Source: CAD feature listing. Evaluate the final solid. Frame: model axes, mm. A direction names the side the tool comes from. Coordinates: 2 decimals unless noted, no trailing zeros. Write each loop counter-clockwise with the first axis right and the second up, starting at its lowest first coordinate (ties: lowest second). Pieces come first, ordered by that corner, then holes. Notation, with made-up numbers: (2, 22) -> (14, 22) arc R30 ccw to (14, 55) -> close; hole circle Ø5 at (29.25, -3.75). An arc over 180 degrees is marked (long way). One line per item, written item: value. Start each with the question number.
1. Section query A-A, the plane y = 127.5. Output: boundary loops of the cut face in (x, z), and give its area (3 significant figures).
2. First-contact query: P1, Ø1.3, axis at y = -17.5, z = 23, coming from the -X side; P2, Ø2, axis at y = -14.5, z = 23.5, coming from the +X side; P3, Ø4.5, axis at x = 36.77, z = 36.77, coming from the -Y side. Flat tips, straight axial feed; report the tip coordinate or a pass-through.
3. Mould query, pull axis X, two halves, no side actions, for faces 1 (the flat face through (-1, 24, 45)), 2 (the conical face through (-36.75, 18.241, -37.203)), 3 (the cylindrical face through (-17.235, 104.695, 41.569)), 4 (the conical face through (-37.203, 18.241, 36.75)). Classes: released by +X, released by -X, zero draft, split by the parting line, or undercut.
4. Access query for faces 5 (the flat face through (-30, 163, 13)), 6 (the flat face through (0, -18, 22.5)), 7 (the flat face through (-34, 48, 34)), 8 (the flat face through (-34, 48, -34)). Directions: +Z, -Z, +X, -X, +Y, -Y. A direction counts if a zero-diameter tool reaches every point of the face in a straight line with its end or side. Return the directions, or none.
5. Line query: line 1 (Y direction, x = 25, z = 14); line 2 (Y direction, x = 29.5, z = -32); line 3 (X direction, y = 130, z = 0.5). Output: solid intervals per line, ascending.
from build123d import *

# Parameters (mm, degrees)
SKETCH_1_W               = 90
SKETCH_1_H               = 90
EXTRUDE_1_DEPTH          = 43
SKETCH_2_R               = 18
EXTRUDE_2_DEPTH          = 3
SKETCH_3_R               = 7.5
EXTRUDE_3_DEPTH          = 29
CUT_EXTRUDE_1_DEPTH      = 3
PATTERN_CIRCULAR_1_COUNT = 4
SKETCH_8_R               = 45
EXTRUDE_4_DEPTH          = 120
SKETCH_9_R               = 32.5
EXTRUDE_5_DEPTH          = 5
SKETCH_10_W              = 90
SKETCH_10_H              = 90
EXTRUDE_6_DEPTH          = 5
FILLET_1_R               = 5
FILLET_2_R               = 2


with BuildPart() as part:
    # 草图1 → 凸台-拉伸1 (new body)
    with BuildSketch(Plane(origin=(0, 0, 0), x_dir=(1, 0, 0), z_dir=(0, 1, 0))):
        Rectangle(SKETCH_1_W, SKETCH_1_H)
    extrude(amount=EXTRUDE_1_DEPTH)

    # 草图2 → 凸台-拉伸2 (add)
    with BuildSketch(Plane.XZ):
        with Locations(Location((0, 18, 0), (0, 0, 90))):
            Circle(SKETCH_2_R)
    extrude(amount=EXTRUDE_2_DEPTH)

    # 草图3 → 凸台-拉伸3 (add)
    with BuildSketch(Plane.XZ.offset(3)):
        with Locations(Location((0, 18, 0), (0, 0, 90))):
            Circle(SKETCH_3_R)
    extrude(amount=EXTRUDE_3_DEPTH)

    # 草图4 → 切除-拉伸1 (cut)
    with BuildSketch(Plane.XY.offset(25.5)):
        with BuildLine():
            Line((-2.5, -7), (-2.5, -32))
            Line((-2.5, -32), (2.5, -32))
            Line((2.5, -32), (2.5, -7))
            ThreePointArc((2.5, -7), (0, -4.5), (-2.5, -7))
        make_face()
    extrude(amount=-CUT_EXTRUDE_1_DEPTH, mode=Mode.SUBTRACT)

    # 草图6 → M6x1.0 螺纹孔1 (revolve, cut)
    with BuildSketch(Plane(origin=(36.769552622, 0, 36.769552622), x_dir=(0, 0, -1), z_dir=(1, 0, 0))):
        Polygon((0, 0), (0, 18.502151548), (2.5, 17), (2.5, 0), align=None)
    m6x1_0_1 = revolve(axis=Axis((36.769552622, -6.35, 36.769552622), (0, 1, 0)), mode=Mode.SUBTRACT)

    # 阵列(圆周)1: M6x1.0 螺纹孔1 ×4 about axis
    pattern_circular_1_axis = Axis((0, 0, 0), (0, 1, 0))
    for i in range(1, PATTERN_CIRCULAR_1_COUNT):
        add(m6x1_0_1.rotate(pattern_circular_1_axis, i * 360 / PATTERN_CIRCULAR_1_COUNT), mode=Mode.SUBTRACT)

    # 草图8 → 凸台-拉伸4 (add)
    with BuildSketch(Plane(origin=(0, 43, 0), x_dir=(1, 0, 0), z_dir=(0, 1, 0))):
        with Locations(Location((0, 0, 0), (0, 0, 270))):
            Circle(SKETCH_8_R)
    extrude(amount=EXTRUDE_4_DEPTH)

    # 草图9 → 凸台-拉伸5 (add)
    with BuildSketch(Plane(origin=(0, 163, 0), x_dir=(1, 0, 0), z_dir=(0, 1, 0))):
        with Locations(Location((0, 0, 0), (0, 0, 270))):
            Circle(SKETCH_9_R)
    extrude(amount=EXTRUDE_5_DEPTH)

    # 草图10 → 凸台-拉伸6 (add)
    with BuildSketch(Plane(origin=(0, 43, 0), x_dir=(1, 0, 0), z_dir=(0, 1, 0))):
        Rectangle(SKETCH_10_W, SKETCH_10_H)
    extrude(amount=EXTRUDE_6_DEPTH)

    # 圆角1
    fillet_1_edges = [part.edges().sort_by_distance(p)[0] for p in [
        (-45, 24, -45),
        (45, 24, -45),
        (45, 24, 45),
        (-45, 24, 45),
    ]]
    fillet(fillet_1_edges, radius=FILLET_1_R)

    # 圆角2
    fillet_2_edges = [part.edges().sort_by_distance(p)[0] for p in [
        (0, 168, -32.5),
    ]]
    fillet(fillet_2_edges, radius=FILLET_2_R)


solid = part.part
Computed values:
1. outline: circle Ø90 at (0, 0)
1. area: 6,360 mm²
2. P1: stops at x = -6.11
2. P2: stops at x = 6
2. P3: stops at y = 17.15
3. face 1: zero draft
3. face 2: undercut
3. face 3: split by the parting line
3. face 4: undercut
4. face 5: +Y
4. face 6: +Z, -Y
4. face 7: +Z, -X, +Y
4. face 8: -Z, -X, +Y
5. line 1: y = 0 to 168
5. line 2: y = 0 to 163
5. line 3: x = -45 to 45
